Model file for the job. Use its own axes, mm. Face numbers are marked on the shaded views. A direction names the side the tool comes from. Give positions to 0.01 mm unless a question says otherwise; leave off trailing zeros. Loops run counter-clockwise (first coordinate to the right, second up) from the corner with the lowest first, then second, coordinate; pieces in that order, holes last. Notation, with made-up numbers: M -35,36 L 15,36 A37 cw 15,72 Z; hole C -32,86.25 d3. An arc over 180 degrees is marked long. Answer in a Markdown table with one row per item.
```python
from build123d import *

# Parameters (mm, degrees)
SKETCH1_W               = 26
SKETCH1_H               = 89
BOSS_EXTRUDE1_DEPTH     = 3
SKETCH2_R               = 6.75
SKETCH2_R_2             = 6.25
SKETCH2_W               = 18.5
SKETCH2_H               = 32.5
SKETCH2_W_2             = 17.5
SKETCH2_H_2             = 31.5
CUT_EXTRUDE_THIN1_DEPTH = 1
CUT_EXTRUDE_THIN1_TAPER = 44
SKETCH3_R               = 6.25
BOSS_EXTRUDE2_DEPTH     = 3
FILLET1_R               = 1
CHAMFER1_SIZE           = 1.5
SKETCH4_R               = 3
SKETCH4_R_2             = 2
EXTRUDE_THIN2_DEPTH     = 6
SKETCH5_W               = 21.5
SKETCH5_H               = 65
BOSS_EXTRUDE3_DEPTH     = 19


with BuildPart() as part:
    # Sketch1 → Boss-Extrude1 (new body)
    with BuildSketch(Plane(origin=(0, 0, 0), x_dir=(1, 0, 0), z_dir=(0, 1, 0))):
        Rectangle(SKETCH1_W, SKETCH1_H)
    extrude(amount=BOSS_EXTRUDE1_DEPTH)

    # Sketch2 → Cut-Extrude-Thin1 (cut)
    # profile 1 of 2: a face of its own
    with BuildSketch(Plane(origin=(0, 3, 0), x_dir=(1, 0, 0), z_dir=(0, 1, 0))):
        with Locations((0, -16.5)):
            Circle(SKETCH2_R)
        with Locations((0, -16.5)):
            Circle(SKETCH2_R_2, mode=Mode.SUBTRACT)
    # profile 2 of 2: a face of its own
    with BuildSketch(Plane(origin=(0, 3, 0), x_dir=(1, 0, 0), z_dir=(0, 1, 0))):
        with Locations((0, 12.5)):
            Rectangle(SKETCH2_W, SKETCH2_H)
        with Locations((0, 12.5)):
            Rectangle(SKETCH2_W_2, SKETCH2_H_2, mode=Mode.SUBTRACT)
    extrude(amount=-CUT_EXTRUDE_THIN1_DEPTH, taper=CUT_EXTRUDE_THIN1_TAPER, mode=Mode.SUBTRACT)

    # Sketch3 → Boss-Extrude2 (add)
    with BuildSketch(Plane(origin=(0, 3, 0), x_dir=(1, 0, 0), z_dir=(0, 1, 0))):
        with Locations((0, -16.5)):
            Circle(SKETCH3_R)
    extrude(amount=BOSS_EXTRUDE2_DEPTH)

    # Fillet1
    fillet1_edges = [part.edges().sort_by_distance(p)[0] for p in [
        (-6.25, 6, 16.5),
    ]]
    fillet(fillet1_edges, radius=FILLET1_R)

    # Chamfer1
    chamfer1_edges = [part.edges().sort_by_distance(p)[0] for p in [
        (-13, 3, 0),
        (0, 3, 44.5),
        (13, 3, 0),
        (0, 3, -44.5),
    ]]
    chamfer(chamfer1_edges, length=CHAMFER1_SIZE)

    # Sketch4 → Extrude-Thin2 (add)
    # profile 1 of 2: a face of its own
    with BuildSketch(Plane.XZ):
        with Locations((0, -39.5)):
            Circle(SKETCH4_R)
        with Locations((0, -39.5)):
            Circle(SKETCH4_R_2, mode=Mode.SUBTRACT)
    # profile 2 of 2: a face of its own
    with BuildSketch(Plane.XZ):
        with Locations((0, 39.5)):
            Circle(SKETCH4_R)
        with Locations((0, 39.5)):
            Circle(SKETCH4_R_2, mode=Mode.SUBTRACT)
    extrude(amount=EXTRUDE_THIN2_DEPTH)

    # Sketch5 → Boss-Extrude3 (add)
    with BuildSketch(Plane.XZ):
        Rectangle(SKETCH5_W, SKETCH5_H)
    extrude(amount=BOSS_EXTRUDE3_DEPTH)


solid = part.part
```
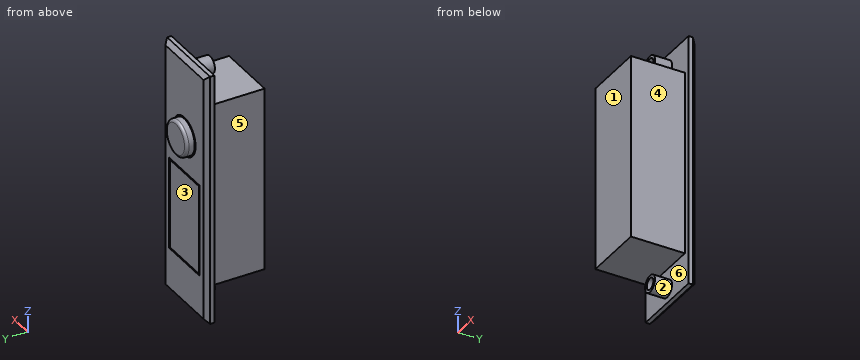
Q1. Probe probe 1 along Z at (x, y) = (0, -3.1); probe 2 along Z at (x, y) = (1.5, -9); probe 3 along Y at (x, z) = (-4.5, -25.5). List the from-to ranges inside material, lowest first.
Reported:
| item | result |
|---|---|
| probe 1 | -42.5 to -41.5, -37.5 to -36.5, -32.5 to 32.5, 36.5 to 37.5, 41.5 to 42.5 |
| probe 2 | -32.5 to 32.5 |
| probe 3 | -19 to 3 |
Q2. Saw through at B-B (z = 39.5). Give the cut face in (x, y).
Reported:
| item | result |
|---|---|
| outline | M -13,0 L -3,0 L -3,-6 L -2,-6 L -2,0 L 2,0 L 2,-6 L 3,-6 L 3,0 L 13,0 L 13,1.5 L 11.5,3 L -11.5,3 L -13,1.5 Z |
Q3. Mould opens along Z. For the marked faces 1 and 2 say: released by +Z, released by -Z, zero draft, split by the parting line, or undercut.
Reported:
| item | result |
|---|---|
| face 1 | zero draft |
| face 2 | undercut |
Q4. Saw through at A-A (y = -2). Give the cut face in (x, z).
Reported:
| item | result |
|---|---|
| outline | M -10.75,-32.5 L 10.75,-32.5 L 10.75,32.5 L -10.75,32.5 Z; C 0,-39.5 d6; C 0,39.5 d6; hole C 0,-39.5 d4; hole C 0,39.5 d4 |
Q5. Saw through at C-C (y = -8.5). Give the cut face in (x, z).
Reported:
| item | result |
|---|---|
| outline | M -10.75,-32.5 L 10.75,-32.5 L 10.75,32.5 L -10.75,32.5 Z |
Q6. Saw through at D-D (z = -35.5). Give the cut face in (x, y).
Reported:
| item | result |
|---|---|
| outline | M -13,0 L 13,0 L 13,1.5 L 11.5,3 L -11.5,3 L -13,1.5 Z |
Q7. 3-axis set-ups, long thin cutter, end or side, ignore diameter. For the marked faces 3, 4, 5 and 6: which of +Z, -Z, +X, -X, +Y, -Y reach the whole face in a straight line?
Reported:
| item | result |
|---|---|
| face 3 | -Z, +X, -X, +Y |
| face 4 | +Z, -Z, +X, -Y |
| face 5 | +Z, -Z, -X, -Y |
| face 6 | -Y |
Q8. Drop flat-ended pins along their axis: pin 1 (7 mm diameter, centred on x = -1.5, z = 1.5, fed in from +Y); pin 2 (5.5 mm diameter, centred on x = -3, y = -11.5, fed in from +Z); pin 3 (5 mm diameter, centred on x = 0, z = 39.5, fed in from -Y); pin 4 (8 mm diameter, centred on x = 1, z = 22.5, fed in from +Y). Give the stop position or say it passes through.
Reported:
| item | result |
|---|---|
| pin 1 | y = 3 |
| pin 2 | z = 32.5 |
| pin 3 | y = -6 |
| pin 4 | y = 6 |
